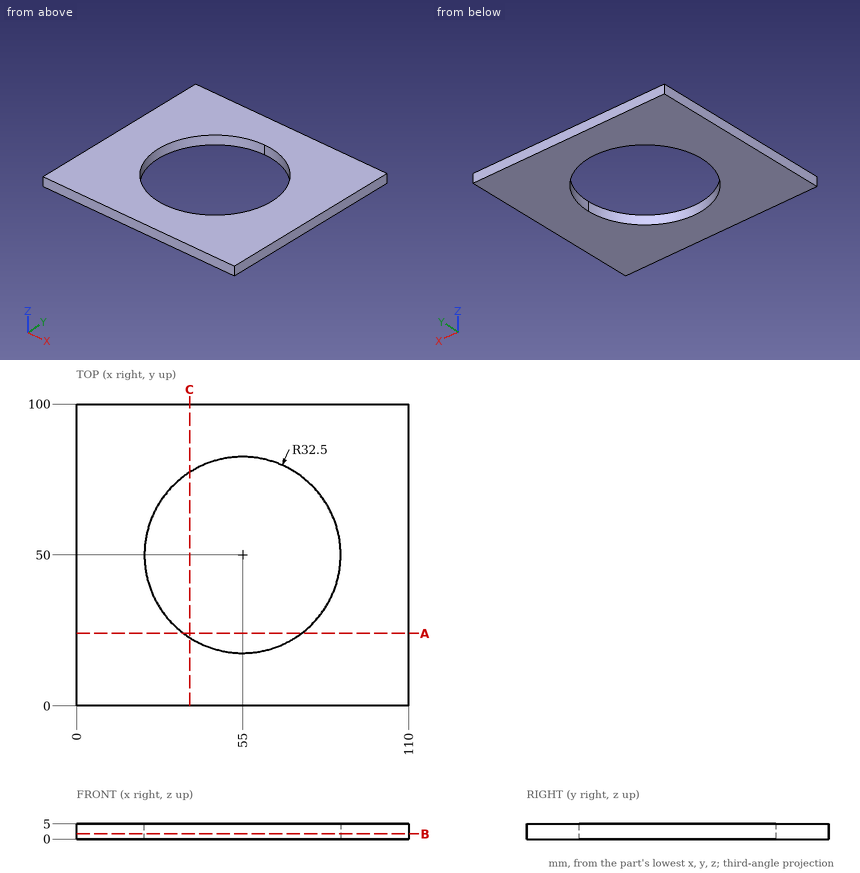
Geometry check sheet. Reference: drawing and pictorial views, mm from the part's lowest x, y, z. Coordinates: 2 decimals unless noted, no trailing zeros. Write each loop counter-clockwise with the first axis right and the second up, starting at its lowest first coordinate (ties: lowest second). Pieces come first, ordered by that corner, then holes. Notation, with made-up numbers: (-22.75, -0.75) -> (-17.75, -0.75) arc R23 ccw to (-17.75, 8.25) -> close; hole circle Ø4 at (32.5, 41.25). An arc over 180 degrees is marked (long way). Use a Markdown table: item, result.
1. Sectioned sample at C-C (x = 37.5). Enter the section's corners in (y, z), plus the area to 3 significant figures.
Reported:
| item | result |
|---|---|
| outline | (0, 0) -> (22.61, 0) -> (22.61, 5) -> (0, 5) -> close; (77.39, 0) -> (100, 0) -> (100, 5) -> (77.39, 5) -> close |
| area | 226 mm2 |
2. Scan lines: line 1 along X through (y, z) = (26, 1.7); line 2 along X through (y, z) = (55, 3.7); line 3 along Y through (x, z) = (43, 0.65). Record each from-to range of solid material in increasing order.
Reported:
| item | result |
|---|---|
| line 1 | x = 0 to 33.09, 76.91 to 110 |
| line 2 | x = 0 to 22.89, 87.11 to 110 |
| line 3 | y = 0 to 19.8, 80.2 to 100 |
3. Sectioned sample at A-A (y = 24). Enter the section's corners in (x, z).
Reported:
| item | result |
|---|---|
| outline | (0, 0) -> (35.5, 0) -> (35.5, 5) -> (0, 5) -> close; (74.5, 0) -> (110, 0) -> (110, 5) -> (74.5, 5) -> close |
4. Sectioned sample at B-B (z = 1.7). Enter the section's corners in (x, y), plus the area to 3 significant figures.
Reported:
| item | result |
|---|---|
| outline | (0, 0) -> (110, 0) -> (110, 100) -> (0, 100) -> close; hole circle Ø65 at (55, 50) |
| area | 7,680 mm2 |
